```python
from build123d import *

# Parameters (mm, degrees)
BOSS_EXTRUDE1_DEPTH = 0.2


with BuildPart() as part:
    # Sketch1 → Boss-Extrude1 (new body)
    with BuildSketch(Plane.XY):
        Polygon((14.2, 1.7), (18.305715448, 4.08), (19.5, 4.08), (19.5, 3.73), (18.4, 3.73), (14.19879989, 0), (0, 0), (0, 1.7), align=None)
    extrude(amount=BOSS_EXTRUDE1_DEPTH)


solid = part.part
```
Here's how the part is built. I have some questions about the finished solid (model axes, mm). Coordinates: 2 decimals unless noted, no trailing zeros. Write each loop counter-clockwise with the first axis right and the second up, starting at its lowest first coordinate (ties: lowest second). Pieces come first, ordered by that corner, then holes. Notation, with made-up numbers: M 48,37 L 62,37 A28 cw 62,71 Z; hole C 58.5,6 d9. An arc over 180 degrees is marked long. Answer as CSV lines item,"result". Start each with the question number.
Q1. Suppose I cut it at A-A, the plane z = 0.1. List the corners of the cut face in (x, y) for me.
Q2. Suppose I cut it at C-C, the plane y = 3.45. List the corners of the cut face in (x, z) for me.
Q3. I need wall thicknesses on probe 1 along Y at (x, z) = (9.25, 0.1); probe 2 along X at (y, z) = (0.6, 0.15); probe 3 along X at (y, z) = (0.7, 0.1). Which ranges of each line are inside material? Lowest first, please. Write a range as [from, to].
Q4. Suppose I cut it at B-B, the plane x = 6. List the corners of the cut face in (y, z) for me, then the cut area to 3 significant figures.
Entries:
1,outline,"M 0,0 L 14.2,0 L 18.4,3.73 L 19.5,3.73 L 19.5,4.08 L 18.31,4.08 L 14.2,1.7 L 0,1.7 Z"
2,outline,"M 17.22,0 L 18.08,0 L 18.08,0.2 L 17.22,0.2 Z"
3,probe 1,"y = [0, 1.7]"
3,probe 2,"x = [0, 14.87]"
3,probe 3,"x = [0, 14.99]"
4,outline,"M 0,0 L 1.7,0 L 1.7,0.2 L 0,0.2 Z"
4,area,"0.340 mm²"
